The listing builds one solid part. Answer for the finished solid, in the listing's coordinates (mm). Face numbers are marked on the shaded views. A direction names the side the tool comes from. Coordinates: 2 decimals unless noted, no trailing zeros. Order: outer loops, then holes, each group sorted by start corner. A loop starts at its lowest first (then second) coordinate and runs counter-clockwise, first axis right, second up. Notation, with made-up numbers: (-31, 62) -> (-16, 62) arc R20 ccw to (-16, 82) -> close; hole circle Ø5 at (61, -22). An arc over 180 degrees is marked (long way). Write item = value, one per line.
from build123d import *

# Parameters (mm, degrees)
EXTRUDE_5_DEPTH     = 30
SKETCH_5_W          = 22
SKETCH_5_H          = 10
CUT_EXTRUDE_7_DEPTH = 41.081973509
SKETCH_6_R          = 4
CUT_EXTRUDE_8_DEPTH = 40.374028275


with BuildPart() as part:
    # 草图1 → 拉伸5 (new body)
    with BuildSketch(Plane.XY):
        with BuildLine():
            Line((7.228416147, 4), (25, 4))
            Line((25, 4), (25, 8))
            Line((25, 8), (9.256881183, 8))
            ThreePointArc((9.256881183, 8), (0, 13.031312217), (-9.256881183, 8))
            Line((-9.256881183, 8), (-25, 8))
            Line((-25, 8), (-25, 4))
            Line((-25, 4), (-7.228416147, 4))
            ThreePointArc((-7.228416147, 4), (0, 9.5), (7.228416147, 4))
        make_face()
    extrude(amount=EXTRUDE_5_DEPTH)

    # 草图5 → 拉伸7 (cut, through all)
    with BuildSketch(Plane.XZ.offset(-4)):
        with Locations((-14, 25)):
            Rectangle(SKETCH_5_W, SKETCH_5_H)
        with Locations((14, 25)):
            Rectangle(SKETCH_5_W, SKETCH_5_H)
    extrude(amount=-CUT_EXTRUDE_7_DEPTH, mode=Mode.SUBTRACT)

    # 草图6 → 拉伸8 (cut, through all)
    with BuildSketch(Plane(origin=(0, 8, 0), x_dir=(1, 0, 0), z_dir=(0, 1, 0))):
        with Locations(Location((-17.128440592, -10, 0), (0, 0, 180))):
            Circle(SKETCH_6_R)
        with Locations(Location((17.128440592, -10, 0), (0, 0, 180))):
            Circle(SKETCH_6_R)
    extrude(amount=-CUT_EXTRUDE_8_DEPTH, mode=Mode.SUBTRACT)


solid = part.part
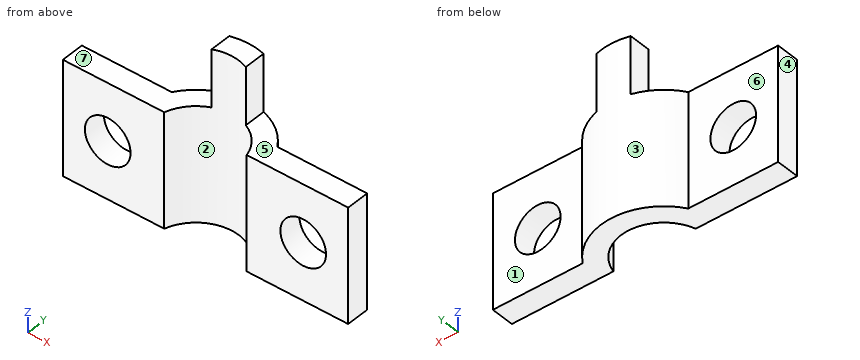
Q1. A tool of negligible diameter and unlimited length cuts with its end or side. For the marked faces 4, 5, 6 and 7, from which of +Z, -Z, +X, -X, +Y, -Y can it reach the whole face along a straight path? Write none if from no direction.
The answers:
face_4 = +Z, -Z, -X, +Y, -Y
face_5 = +Z, +X, +Y, -Y
face_6 = +Z, -Z, -X, +Y
face_7 = +Z, -X, +Y, -Y
Q2. Section B-B, the plane y = 7.25 is taken. Give the vertices of the cut face in (x, z), plus the area to 3 significant figures.
The answers:
outline = (-25, 0) -> (-5.36, 0) -> (-5.36, 20) -> (-25, 20) -> close; (5.36, 0) -> (25, 0) -> (25, 20) -> (5.36, 20) -> close; hole circle Ø8 at (-17.13, 10); hole circle Ø8 at (17.13, 10)
area = 685 mm2
Q3. The mould has two halves that part along X. Classify the marked faces 1, 2 and 3: released by +X, released by -X, zero draft, split by the parting line, or undercut.
The answers:
face_1 = zero draft
face_2 = undercut
face_3 = split by the parting line
Q4. Section C-C, the plane x = -14 is taken. Give the vertices of the cut face in (y, z).
The answers:
outline = (4, 0) -> (8, 0) -> (8, 7.51) -> (4, 7.51) -> close; (4, 12.49) -> (8, 12.49) -> (8, 20) -> (4, 20) -> close
Q5. Each of these flat-tipped pins is pushed along its axis until it touches: pin 1 Ø1 at (x, y) = (-6, 8) entering from +Z; pin 2 Ø2 at (y, z) = (11.5, 5.5) entering from -X; pin 3 Ø12.5 at (x, z) = (20, 6) entering from +Y. Where does it stop, or does it pass through?
The answers:
pin_1 = 20
pin_2 = -7.03
pin_3 = 8
Q6. Find the intervals of material crossed by line 1 along X through (y, z) = (4.5, 9); line 2 along X through (y, z) = (7.5, 13); line 3 along Y through (x, z) = (16, 19), in increasing order.
The answers:
line_1 = -25 to -21, -13.26 to -7.07, 7.07 to 13.26, 21 to 25
line_2 = -25 to -19.77, -14.48 to -5.1, 5.1 to 14.48, 19.77 to 25
line_3 = 4 to 8
Q7. Section A-A, the plane z = 13.5 is taken. Give the vertices of the cut face in (x, y), plus the area to 3 significant figures.
The answers:
outline = (-25, 4) -> (-19.06, 4) -> (-19.06, 8) -> (-25, 8) -> close; (-15.19, 4) -> (-7.23, 4) arc R7.5 cw to (7.23, 4) -> (15.19, 4) -> (15.19, 8) -> (9.26, 8) arc R11.03 ccw to (-9.26, 8) -> (-15.19, 8) -> close; (19.06, 4) -> (25, 4) -> (25, 8) -> (19.06, 8) -> close
area = 176 mm2
Q8. Section D-D, the plane z = 3.75 is taken. Give the vertices of the cut face in (x, y).
The answers:
outline = (-25, 4) -> (-7.23, 4) arc R7.5 cw to (7.23, 4) -> (25, 4) -> (25, 8) -> (9.26, 8) arc R11.03 ccw to (-9.26, 8) -> (-25, 8) -> close
